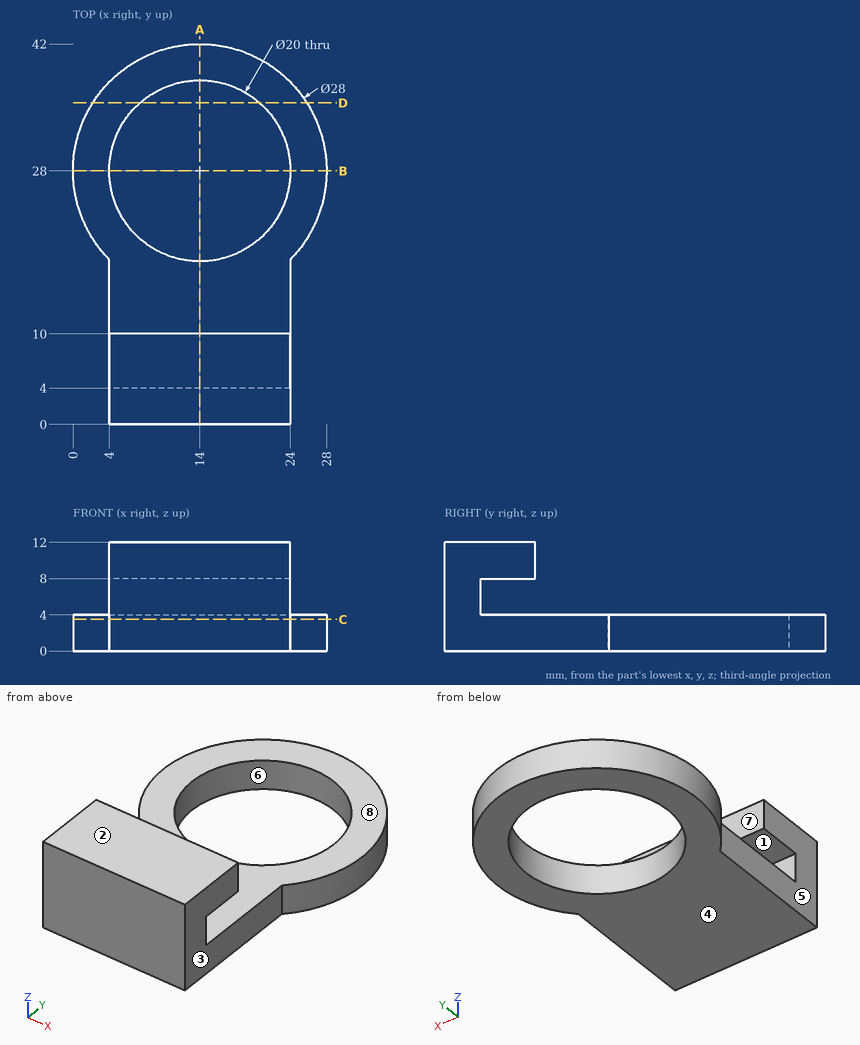
Design review of the part shown in the three views and the two pictorial views. Dimensions are in mm from the part's minimum x, y and z. A direction names the side the tool comes from. Give positions to 0.01 mm unless a question says otherwise; leave off trailing zeros. Write each loop counter-clockwise with the first axis right and the second up, starting at its lowest first coordinate (ties: lowest second). Pieces come first, ordered by that corner, then holes.
Item 1: Insertion check: P1, Ø3.5, axis at y = 7.5, z = 9, coming from the -X side; P2, Ø4, axis at x = 8, y = 13, coming from the +Z side; P3, Ø5, axis at y = 37.5, z = 8, coming from the +X side; P4, Ø1, axis at x = 7, z = 2, coming from the -Y side. Each pin has a flat end and moves straight along its axis. Give the tip position at first contact, or say it passes through.
Item 2: Take a section at B-B (y = 28). Give the boundary of the cut face in (x, z).
Item 3: Wall thickness on probe 1 along Y at (x, z) = (14, 2.45); probe 2 along Z at (x, y) = (26, 26): over which ranges is each line inside the solid? List them lowest first.
Item 4: The part is to be moulded in two halves that separate along Z. For the marked faces 1, 2, 3 and 4, say which applies: +Z half, -Z half, draft (parallel to the pull), parting line (faces both ways), or undercut.
Item 5: Machinability: for the marked faces 5, 6, 7 and 8, which of the approach directions +Z, -Z, +X, -X, +Y, -Y give a long, thin tool a straight path to every point of the face, cutting with its end or side? Answer none if there is none.
Item 6: Take a section at C-C (z = 3.5). Give the boundary of the cut face in (x, y), and give its area (3 significant figures).
Item 7: Take a section at D-D (y = 35.5). Give the boundary of the cut face in (x, z).
Item 8: Take a section at A-A (x = 14). Give the boundary of the cut face in (y, z).
Established:
1. P1: stops at x = 4
1. P2: stops at z = 4
1. P3: passes through
1. P4: stops at y = 0
2. outline: (0, 0) - (4, 0) - (4, 4) - (0, 4) - close; (24, 0) - (28, 0) - (28, 4) - (24, 4) - close
3. probe 1: y = 0 to 18, 38 to 42
3. probe 2: z = 0 to 4
4. face 1: undercut
4. face 2: +Z half
4. face 3: draft
4. face 4: -Z half
5. face 5: +Z, -Z, -X, -Y
5. face 6: +Z, -Z
5. face 7: +Z, +X, -X, +Y
5. face 8: +X, -X, +Y
6. outline: (4, 0) - (24, 0) - (24, 18.2) arc R14 ccw (long way) to (4, 18.2) - close; hole circle Ø20 at (14, 28)
6. area: 608 mm2
7. outline: (2.18, 0) - (7.39, 0) - (7.39, 4) - (2.18, 4) - close; (20.61, 0) - (25.82, 0) - (25.82, 4) - (20.61, 4) - close
8. outline: (0, 0) - (18, 0) - (18, 4) - (4, 4) - (4, 8) - (10, 8) - (10, 12) - (0, 12) - close; (38, 0) - (42, 0) - (42, 4) - (38, 4) - close
